Source: CAD feature listing. Evaluate the final solid. Frame: model axes, mm. A direction names the side the tool comes from. Give positions to 0.01 mm unless a question says otherwise; leave off trailing zeros. Order: outer loops, then holes, each group sorted by start corner. A loop starts at its lowest first (then second) coordinate and runs counter-clockwise, first axis right, second up. Notation, with made-up numbers: (10.5, 25) - (20.5, 25) arc R14 ccw to (20.5, 41) - close; hole circle Ø10 at (-7, 57). An arc over 180 degrees is marked (long way). Answer as CSV lines item,"result".
```python
from build123d import *

# Parameters (mm, degrees)
GB_T6728_2002_40_X_40_X_4_1_DEPTH = 105
HOLE_WIZARD_12_0_12_1_D           = 12
HOLE_WIZARD_12_0_12_1_DEPTH       = 41.394836286
HOLE_WIZARD_12_0_12_1_TIP         = 3.605163714
CUT_EXTRUDE_1_REACH               = 116.127
SKETCH_5_R                        = 8.5


with BuildPart() as part:
    # Sketch1 → 冷弯空心方管gb∕t6728-2002 40 X 40 X 4(1) (new body)
    with BuildSketch(Plane.YZ):
        with BuildLine():
            Line((-12, -20), (12, -20))
            ThreePointArc((12, -20), (17.656854249, -17.656854249), (20, -12))
            Line((20, -12), (20, 12))
            ThreePointArc((20, 12), (17.656854249, 17.656854249), (12, 20))
            Line((12, 20), (-12, 20))
            ThreePointArc((-12, 20), (-17.656854249, 17.656854249), (-20, 12))
            Line((-20, 12), (-20, -12))
            ThreePointArc((-20, -12), (-17.656854249, -17.656854249), (-12, -20))
        make_face()
        with BuildLine():
            Line((-12, -16), (12, -16))
            ThreePointArc((12, -16), (14.828427125, -14.828427125), (16, -12))
            Line((16, -12), (16, 12))
            ThreePointArc((16, 12), (14.828427125, 14.828427125), (12, 16))
            Line((12, 16), (-12, 16))
            ThreePointArc((-12, 16), (-14.828427125, 14.828427125), (-16, 12))
            Line((-16, 12), (-16, -12))
            ThreePointArc((-16, -12), (-14.828427125, -14.828427125), (-12, -16))
        make_face(mode=Mode.SUBTRACT)
    extrude(amount=GB_T6728_2002_40_X_40_X_4_1_DEPTH)

    # Ø12.0 (12) 直径孔1
    with Locations(Plane(origin=(0, 20, 0), x_dir=(1, 0, 0), z_dir=(0, 1, 0))):
        with Locations((16, 0), (89, 0)):
            Hole(HOLE_WIZARD_12_0_12_1_D / 2, depth=HOLE_WIZARD_12_0_12_1_DEPTH)
            with Locations((0, 0, -(HOLE_WIZARD_12_0_12_1_DEPTH + HOLE_WIZARD_12_0_12_1_TIP / 2))):  # 118° drill point
                Cone(0, HOLE_WIZARD_12_0_12_1_D / 2, HOLE_WIZARD_12_0_12_1_TIP, mode=Mode.SUBTRACT)

    # 切除-拉伸1: up to this face of the body (flat: up to its plane)
    cut_extrude_1_end = Plane(part.part.faces().sort_by_distance((52.5, 0, 20))[0])
    # 草图5 → 切除-拉伸1 (cut, up to the picked face)
    with BuildSketch(Plane(origin=(0, 0, -20), x_dir=(-1, 0, 0), z_dir=(0, 0, -1)), mode=Mode.PRIVATE) as cut_extrude_1_sk1:
        with Locations((-52.5, 0)):
            Circle(SKETCH_5_R)
    cut_extrude_1_tool1 = split(extrude(cut_extrude_1_sk1.sketch, amount=-CUT_EXTRUDE_1_REACH, mode=Mode.PRIVATE), bisect_by=cut_extrude_1_end, keep=Keep.BOTH, mode=Mode.PRIVATE)
    add(cut_extrude_1_tool1.solids().sort_by(Axis((52.5, 0, -20), (0, 0, 1)))[0], mode=Mode.SUBTRACT)


solid = part.part
```
(1) Mould query, pull axis Z, two halves, no side actions, for faces 1 (the cylindrical face through (51.765, -14.859, -14.797)), 2 (the flat face through (52, 10, -20)), 3 (the cylindrical face through (61, 0, -18)). Classes: released by +Z, released by -Z, zero draft, split by the parting line, or undercut.
Completed:
face 1,"undercut"
face 2,"released by -Z"
face 3,"zero draft"
(2) Ray query, line 1 (Z direction, x = 51.5, y = -12); line 2 (X direction, y = -18, z = -4). Return the intervals inside material, ascending. Write a range as from..to.
Completed:
line 1,"-20..-16, 16..20"
line 2,"0..11.53, 20.47..84.53, 93.47..105"
(3) Cut plane D-D (y = -10.5). Return loops of the section in (x, z).
Completed:
outline,"(0, -20) - (105, -20) - (105, -16) - (0, -16) - close; (0, 16) - (105, 16) - (105, 20) - (0, 20) - close"
(4) Cut plane C-C (z = 0). Return loops of the section in (x, y), then the cut area to 3 significant figures.
Completed:
outline,"(0, -20) - (10, -20) - (10, -16) - (0, -16) - close; (0, 16) - (10, 16) - (10, 20) - (0, 20) - close; (22, -20) - (83, -20) - (83, -16) - (22, -16) - close; (22, 16) - (83, 16) - (83, 20) - (22, 20) - close; (95, -20) - (105, -20) - (105, -16) - (95, -16) - close; (95, 16) - (105, 16) - (105, 20) - (95, 20) - close"
area,"648 mm²"
(5) Cut plane A-A (y = 0). Return loops of the section in (x, z), then the cut area to 3 significant figures.
Completed:
outline,"(0, -20) - (44, -20) - (44, -16) - (0, -16) - close; (0, 16) - (44, 16) - (44, 20) - (0, 20) - close; (61, -20) - (105, -20) - (105, -16) - (61, -16) - close; (61, 16) - (105, 16) - (105, 20) - (61, 20) - close"
area,"704 mm²"
(6) Access query for faces 4 (the flat face through (52, -10, 16)), 5 (the flat face through (52, -10, 20)). Directions: +Z, -Z, +X, -X, +Y, -Y. A direction counts if a zero-diameter tool reaches every point of the face in a straight line with its end or side. Return the directions, or none.
Completed:
face 4,"+X, -X"
face 5,"+Z, +X, -X, +Y, -Y"
(7) Cut plane B-B (x = 89). Return loops of the section in (y, z), then the cut area to 3 significant figures.
Completed:
outline,"(-20, -12) arc R8 ccw to (-12, -20) - (12, -20) arc R8 ccw to (20, -12) - (20, -6) - (16, -6) - (16, -12) arc R4 cw to (12, -16) - (-12, -16) arc R4 cw to (-16, -12) - (-16, -6) - (-20, -6) - close; (-20, 6) - (-16, 6) - (-16, 12) arc R4 cw to (-12, 16) - (12, 16) arc R4 cw to (16, 12) - (16, 6) - (20, 6) - (20, 12) arc R8 ccw to (12, 20) - (-12, 20) arc R8 ccw to (-20, 12) - close"
area,"439 mm²"
